Read the model definition and answer for the solid it produces. Units are mm, in the model's axes. A direction names the side the tool comes from. Coordinates: 2 decimals unless noted, no trailing zeros. Write each loop counter-clockwise with the first axis right and the second up, starting at its lowest first coordinate (ties: lowest second). Pieces come first, ordered by that corner, then holes.
(1) The part is cut by section D-D, the plane x = -19.5. Determine the outline of the cut face in (y, z), and give its area (3 significant figures).
(2) Which of the six approach directions +Z, -Z, +X, -X, +Y, -Y give full straight-line access (tool end or side, diameter ignored) to faces 1 (the flat face through (-26, 0, 0)), 2 (the cylindrical face through (19.59, -0.54, 2.44)), 3 (the flat face through (-13, -2, -2))?
(3) The part is cut by section C-C, the plane x = 8. Determine the outline of the cut face in (y, z).
(4) Straight lines are drawn through the part: line 1 along X through (y, z) = (1.25, -3.5); line 2 along Y through (x, z) = (-3.5, 1); line 3 along Z through (x, y) = (3, -1.5). For each, find the intervals that lie inside material, in ascending order.
(5) The part is cut by section A-A, the plane z = 0. Determine the outline of the cut face in (x, y), and give its area (3 significant figures).
(6) Given pin 1 (2 mm diameter, centred on x = 1.5, z = 1, fed in from -Y); pin 2 (1 mm diameter, centred on y = 1.5, z = 3, fed in from +X), each flat-ended and moving along its own axis, determine where each tip first touches the part or whether it passes through.
```python
from build123d import *


with BuildPart() as part:
    # Sketch1 → Revolve1 (revolve)
    with BuildSketch(Plane.XY):
        Polygon((26, 0), (-26, 0), (-26, 2.5), (-13, 2.5), (-13, 4), (13, 4), (13, 2.5), (26, 2.5), align=None)
    revolve(axis=Axis((26, 0, 0), (-1, 0, 0)))


solid = part.part
```
Computed:
1. outline: circle Ø5 at (0, 0)
1. area: 19.6 mm2
2. face 1: +Z, -Z, -X, +Y, -Y
2. face 2: +X
2. face 3: -X
3. outline: circle Ø8 at (0, 0)
4. line 1: x = -13 to 13
4. line 2: y = -3.87 to 3.87
4. line 3: z = -3.71 to 3.71
5. outline: (-26, -2.5) - (-13, -2.5) - (-13, -4) - (13, -4) - (13, -2.5) - (26, -2.5) - (26, 2.5) - (13, 2.5) - (13, 4) - (-13, 4) - (-13, 2.5) - (-26, 2.5) - close
5. area: 338 mm2
6. pin 1: stops at y = -4
6. pin 2: stops at x = 13
